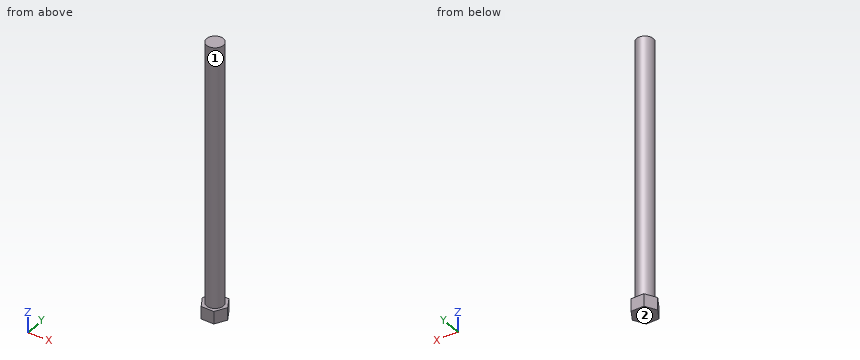
```python
from build123d import *

# Parameters (mm, degrees)
SKETCH_1_R      = 8
EXTRUDE_1_DEPTH = 250
EXTRUDE_2_DEPTH = 12


with BuildPart() as part:
    # 草图1 → 凸台-拉伸1 (new body)
    with BuildSketch(Plane.XY):
        Circle(SKETCH_1_R)
    extrude(amount=EXTRUDE_1_DEPTH)

    # 草图2 → 凸台-拉伸2 (add)
    with BuildSketch(Plane.XY):
        Polygon((12, 0), (6, 10.392304845), (-6, 10.392304845), (-12, 0), (-6, -10.392304845), (6, -10.392304845), align=None)
    extrude(amount=-EXTRUDE_2_DEPTH)


solid = part.part
```
The listing builds one solid part. Answer for the finished solid, in the listing's coordinates (mm). Face numbers are marked on the shaded views. A direction names the side the tool comes from. Round coordinates to 2 decimals unless told otherwise and drop trailing zeros. Loops run counter-clockwise (first coordinate to the right, second up) from the corner with the lowest first, then second, coordinate; pieces in that order, holes last. Notation, with made-up numbers: (87, 46) - (91, 46) arc R34 cw to (91, 76) - close; hole circle Ø9 at (69.5, 84). An arc over 180 degrees is marked (long way). Return JSON: item names as keys, results as strings. Group by question number.
1. The part is cut by section A-A on x = 0. Determine the outline of the cut face in (y, z).
2. Each of these flat-tipped pins is pushed along its axis until it touches: P1, Ø8, axis at y = -8, z = 39, coming from the -X side; P2, Ø2, axis at x = 7, y = 6, coming from the +Z side; P3, Ø3, axis at x = -7, z = 177, coming from the +Y side. Where does it stop, or does it pass through?
3. The part is cut by section C-C on z = 202.5. Determine the outline of the cut face in (x, y), then the cut area to 3 significant figures.
4. Which of the six approach directions +Z, -Z, +X, -X, +Y, -Y give full straight-line access (tool end or side, diameter ignored) to the marked faces 1 and 2?
5. The part is cut by section B-B on y = -4.25. Determine the outline of the cut face in (x, z).
6. Consider probe 1 along Z at (x, y) = (-9.25, 1.5); probe 2 along X at (y, z) = (4.25, 93.5); probe 3 along X at (y, z) = (-3.5, 16). Determine where each line is inside the solid, lowest interval first.
Resolved:
{
 "1": {"outline": "(-10.39, -12) - (10.39, -12) - (10.39, 0) - (8, 0) - (8, 250) - (-8, 250) - (-8, 0) - (-10.39, 0) - close"},
 "2": {"P1": "stops at x = -6.93", "P2": "stops at z = 0", "P3": "stops at y = 5.81"},
 "3": {"outline": "circle Ø16 at (0, 0)", "area": "201 mm²"},
 "4": {"face 1": "+Z", "face 2": "-Z, +X, -X, +Y, -Y"},
 "5": {"outline": "(-9.55, -12) - (9.55, -12) - (9.55, 0) - (6.78, 0) - (6.78, 250) - (-6.78, 250) - (-6.78, 0) - (-9.55, 0) - close"},
 "6": {"probe 1": "z = -12 to 0", "probe 2": "x = -6.78 to 6.78", "probe 3": "x = -7.19 to 7.19"}
}
